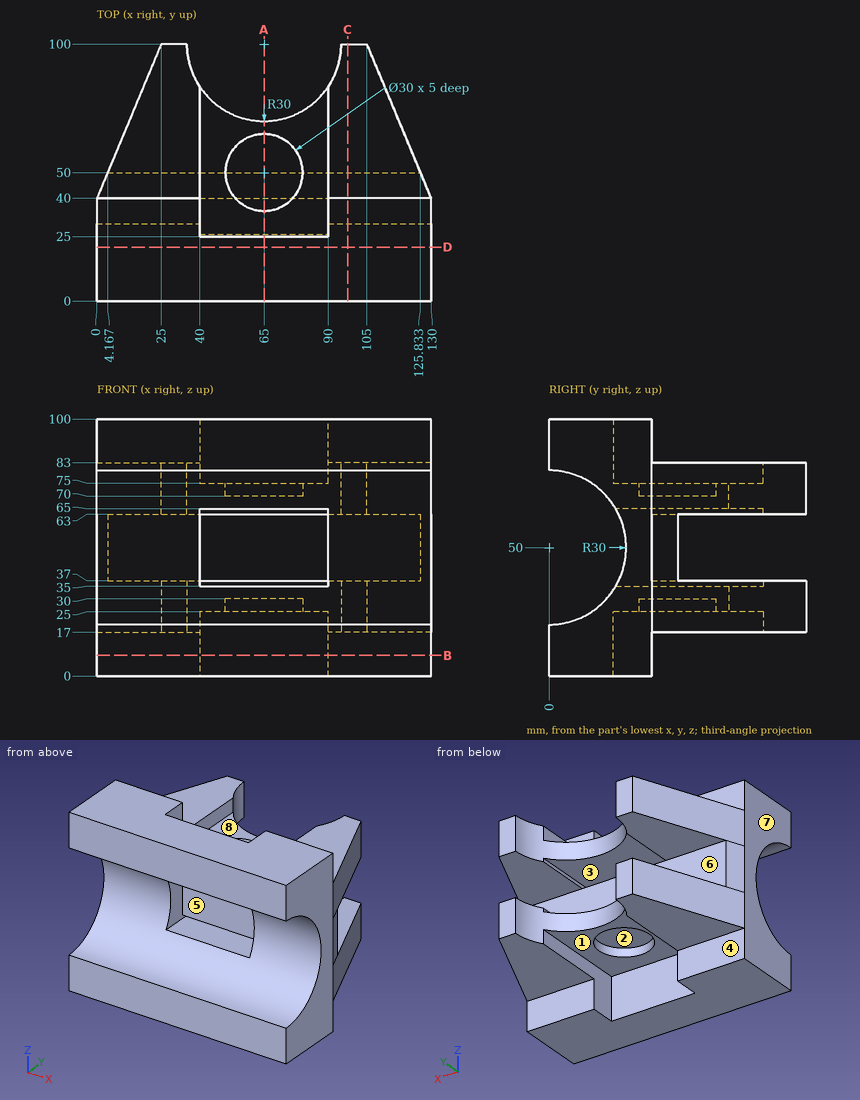
Could you check a few things on this drawing? It's one solid part, dimensions in mm from its lowest x, y, z. A direction names the side the tool comes from. Round coordinates to 2 decimals unless told otherwise and drop trailing zeros. Write each loop counter-clockwise with the first axis right and the second up, starting at its lowest first coordinate (ties: lowest second). Pieces come first, ordered by that corner, then holes. Notation, with made-up numbers: (58, 61) -> (74, 61) arc R24 ccw to (74, 87) -> close; hole circle Ø9 at (85, -27.75). An arc over 180 degrees is marked (long way). Use one line per item in the form item = value. Start each with the question number.
Q1. Imagine slicing it at C-C (x = 97.5). Please give me the cut outline in (y, z), then the cut area to 3 significant figures.
Q2. Imagine slicing it at A-A (x = 65). Please give me the cut outline in (y, z).
Q3. If I drill on probe 1 along Z at (x, y) = (76, 47.5); probe 2 along Z at (x, y) = (79.5, 52); probe 3 along Z at (x, y) = (89.5, 34.5), over which ranges is the centre line in solid material (lowest first)? Write a range as [from, to].
Q4. Imagine slicing it at D-D (y = 21). Please give me the cut outline in (x, z), then the cut area to 3 significant figures.
Q5. Which directions (+Z, -Z, +X, -X, +Y, -Y) give clear straight access to the entire face, cutting with the end or side of a thin tool? Please do the marked faces 1, 2, 3, 4 and 5.
Q6. Imagine slicing it at B-B (z = 8). Please give me the cut outline in (x, y), then the cut area to 3 significant figures.
Q7. I'm going to push flat-ended pins straight in: P1, Ø8, axis at x = 60, y = 45, coming from the +Z side; P2, Ø8, axis at x = 56.5, z = 50, coming from the -Y side; P3, Ø12.5, axis at y = 57.5, z = 86.5, coming from the -X side (1 decimal). Where does each tip first touch, or does it pass through?
Q8. We'd pull the mould along X, two halves only. Please class the marked faces 6, 7 and 8: +X half, -X half, draft (parallel to the pull), parting line (faces both ways), or undercut.
Worked out:
q1.outline = (0, 0) -> (40, 0) -> (40, 17) -> (100, 17) -> (100, 37) -> (50, 37) -> (50, 63) -> (100, 63) -> (100, 83) -> (40, 83) -> (40, 100) -> (0, 100) -> (0, 80) arc R30 cw to (0, 20) -> close
q1.area = 5,250 mm^2
q2.outline = (0, 0) -> (25, 0) -> (25, 25) -> (35, 25) -> (35, 30) -> (65, 30) -> (65, 25) -> (70, 25) -> (70, 35) -> (25.98, 35) arc R30 cw to (0, 20) -> close; (0, 80) arc R30 cw to (25.98, 65) -> (70, 65) -> (70, 75) -> (65, 75) -> (65, 70) -> (35, 70) -> (35, 75) -> (25, 75) -> (25, 100) -> (0, 100) -> close; (40, 37) -> (50, 37) -> (50, 63) -> (40, 63) -> close
q3.probe_1 = [30, 35], [37, 63], [65, 70]
q3.probe_2 = [30, 35], [65, 70]
q3.probe_3 = [25, 35], [65, 75]
q4.outline = (0, 0) -> (130, 0) -> (130, 28.58) -> (0, 28.58) -> close; (0, 71.42) -> (130, 71.42) -> (130, 100) -> (0, 100) -> close
q4.area = 7,430 mm^2
q5.face_1 = -Z, +Y
q5.face_2 = -Z
q5.face_3 = +Y, -Y
q5.face_4 = -Z, +X, -X, +Y
q5.face_5 = -Y
q6.outline = (0, 0) -> (130, 0) -> (130, 40) -> (90, 40) -> (90, 25) -> (40, 25) -> (40, 40) -> (0, 40) -> close
q6.area = 4,450 mm^2
q7.P1 = 70
q7.P2 = 40
q7.P3 = 5.1
q8.face_6 = draft
q8.face_7 = -X half
q8.face_8 = undercut
